from build123d import *

# Parameters (mm, degrees)
SKETCH_1_W              = 185
SKETCH_1_H              = 40.883977901
EXTRUDE_1_DEPTH         = 34
SKETCH_2_W              = 100
SKETCH_2_H              = 30
CUT_EXTRUDE_1_DEPTH     = 192.824137295
SKETCH_3_W              = 81
SKETCH_3_H              = 30
CUT_EXTRUDE_2_DEPTH     = 192.824137295
CUT_EXTRUDE_3_DEPTH     = 193.490258582
CUT_EXTRUDE_4_DEPTH     = 192.824137295
HOLE_WIZARD_18_0_18_1_D = 18
CHAMFER_1_SIZE          = 5
FILLET_1_R              = 2
FILLET_2_R              = 6


with BuildPart() as part:
    # 草图1 → 凸台-拉伸1 (new body)
    with BuildSketch(Plane.XZ.offset(30)):
        with Locations((92.5, 20.441988951)):
            Rectangle(SKETCH_1_W, SKETCH_1_H)
    extrude(amount=-EXTRUDE_1_DEPTH)

    # 草图2 → 切除-拉伸1 (cut, through all)
    with BuildSketch(Plane(origin=(0, 0, 0), x_dir=(-1, 0, 0), z_dir=(0, 0, -1))):
        with Locations((-135, -11)):
            Rectangle(SKETCH_2_W, SKETCH_2_H)
    extrude(amount=-CUT_EXTRUDE_1_DEPTH, mode=Mode.SUBTRACT)

    # 草图3 → 切除-拉伸2 (cut, through all)
    with BuildSketch(Plane(origin=(0, 0, 0), x_dir=(-1, 0, 0), z_dir=(0, 0, -1))):
        with Locations((-40.5, -15)):
            Rectangle(SKETCH_3_W, SKETCH_3_H)
    extrude(amount=-CUT_EXTRUDE_2_DEPTH, mode=Mode.SUBTRACT)

    # 草图4 → 切除-拉伸3 (cut, through all)
    with BuildSketch(Plane.XZ.offset(30)):
        with BuildLine():
            Line((171, 13.5), (151, 13.5))
            ThreePointArc((151, 13.5), (147.5, 10), (151, 6.5))
            Line((151, 6.5), (171, 6.5))
            ThreePointArc((171, 6.5), (174.5, 10), (171, 13.5))
        make_face()
    extrude(amount=-CUT_EXTRUDE_3_DEPTH, mode=Mode.SUBTRACT)

    # 草图5 → 切除-拉伸4 (cut, through all)
    with BuildSketch(Plane(origin=(0, -26, 0), x_dir=(-1, 0, 0), z_dir=(0, 1, 0))):
        with BuildLine():
            Line((-151, 33.5), (-171, 33.5))
            ThreePointArc((-171, 33.5), (-174.5, 30), (-171, 26.5))
            Line((-171, 26.5), (-151, 26.5))
            ThreePointArc((-151, 26.5), (-147.5, 30), (-151, 33.5))
        make_face()
    extrude(amount=-CUT_EXTRUDE_4_DEPTH, mode=Mode.SUBTRACT)

    # Ø18.0 (18) 直径孔1 (through all)
    with Locations(Plane(origin=(0, 0, 0), x_dir=(-1, 0, 0), z_dir=(0, -1, 0))):
        with Locations((-15, -20)):
            Hole(HOLE_WIZARD_18_0_18_1_D / 2)

    # 倒角1
    chamfer_1_edges = [part.edges().sort_by_distance(p)[0] for p in [
        (185, -28, 0),
        (185, -28, 40.883977901),
        (0, 2, 40.883977901),
        (0, 2, 0),
    ]]
    chamfer(chamfer_1_edges, length=CHAMFER_1_SIZE)

    # 圆角1
    fillet_1_edges = [part.edges().sort_by_distance(p)[0] for p in [
        (85, -26, 20.44198895),
        (81, 0, 20.44198895),
    ]]
    fillet(fillet_1_edges, radius=FILLET_1_R)

    # 圆角2
    fillet_2_edges = [part.edges().sort_by_distance(p)[0] for p in [
        (85, 4, 20.44198895),
        (81, -30, 20.44198895),
    ]]
    fillet(fillet_2_edges, radius=FILLET_2_R)


solid = part.part
Design review of the part built by this model. Coordinates are the model's own, in mm. A direction names the side the tool comes from. Coordinates: 2 decimals unless noted, no trailing zeros. Write each loop counter-clockwise with the first axis right and the second up, starting at its lowest first coordinate (ties: lowest second). Pieces come first, ordered by that corner, then holes. Notation, with made-up numbers: (32.5, 43.25) - (59.5, 43.25) arc R27 ccw to (59.5, 66.25) - close; hole circle Ø3 at (-28.5, 74). An arc over 180 degrees is marked (long way). One line per item, written item: value.
1) For faces 4 (the face through (2.535, 1.972, 38.419)), 5 (the face through (81, -13, 20)), 6 (the face through (147.5, -28, 10.1)), list the 3-axis set-ups (+Z, -Z, +X, -X, +Y, -Y) from which the entire face can be reached by the end or side of a thin tool; tool diameter is ignored.
Answer sheet:
face 4: +Z, -X, +Y, -Y
face 5: +Z, -Z, -X, -Y
face 6: +Y, -Y
2) Mouldability with a two-part tool opening along X and no side actions: class faces 1 (the face through (182.535, -28.028, 38.349)), 2 (the face through (92, -27, 40.884)), 3 (the face through (161, -28, 26.5)) as +X half, -X half, draft (parallel to the pull), parting line (faces both ways), or undercut.
Answer sheet:
face 1: +X half
face 2: draft
face 3: undercut
3) Add section D-D (x = 34). State the section outline as (y, z) points.
Answer sheet:
outline: (0, 0) - (4, 0) - (4, 40.88) - (0, 40.88) - close
4) Add section A-A (x = 15). State the section outline as (y, z) points, plus the area to 3 significant figures.
Answer sheet:
outline: (0, 0) - (4, 0) - (4, 11) - (0, 11) - close; (0, 29) - (4, 29) - (4, 40.88) - (0, 40.88) - close
area: 91.5 mm2
5) Insertion check: pin 1 (12.5 mm diameter, centred on x = 130, z = 23.5, fed in from +Y); pin 2 (4 mm diameter, centred on x = 75.5, z = 27, fed in from -Y); pin 3 (3 mm diameter, centred on y = -16, z = 12.5, fed in from -X). Each pin has a flat end and moves straight along its axis. Give the tip position at first contact, or say it passes through.
Answer sheet:
pin 1: stops at y = -26
pin 2: stops at y = 0
pin 3: stops at x = 81
6) To check wall thickness, follow probe 1 along Y at (x, z) = (88, 3); probe 2 along Z at (x, y) = (15, 2.45); probe 3 along Y at (x, z) = (35, 24). State the ranges of each line that lie inside material, in increasing order.
Answer sheet:
probe 1: y = -30 to -26
probe 2: z = 0 to 11, 29 to 40.88
probe 3: y = 0 to 4
7) Add section C-C (y = -14). State the section outline as (x, z) points.
Answer sheet:
outline: (81, 0) - (85, 0) - (85, 40.88) - (81, 40.88) - close
8) Add section B-B (z = 20). State the section outline as (x, y) points.
Answer sheet:
outline: (0, 0) - (6, 0) - (6, 4) - (0, 4) - close; (24, 0) - (79, 0) arc R2 cw to (81, -2) - (81, -24) arc R6 ccw to (87, -30) - (185, -30) - (185, -26) - (87, -26) arc R2 cw to (85, -24) - (85, -2) arc R6 ccw to (79, 4) - (24, 4) - close
